Source: CAD feature listing. Evaluate the final solid. Frame: model axes, mm. A direction names the side the tool comes from. Coordinates: 2 decimals unless noted, no trailing zeros. Order: outer loops, then holes, each group sorted by start corner. A loop starts at its lowest first (then second) coordinate and runs counter-clockwise, first axis right, second up. Notation, with made-up numbers: (-10.75, -9) -> (28.25, -9) arc R20 cw to (28.25, 18) -> close; hole circle Ø10 at (-31.5, -36.5). An arc over 180 degrees is marked (long way). Put each result on its own line as item: value.
from build123d import *

# Parameters (mm, degrees)
BOSS_EXTRUDE1_DEPTH = 100
SKETCH2_R           = 10
CUT_EXTRUDE1_DEPTH  = 500
CUT_EXTRUDE2_DEPTH  = 500


with BuildPart() as part:
    # Sketch1 → Boss-Extrude1 (new body)
    with BuildSketch(Plane.XY):
        Polygon((0, 0), (100, 0), (100, -15), (-15, -15), (-15, 95), (100, 95), (100, 80), (0, 80), align=None)
    extrude(amount=BOSS_EXTRUDE1_DEPTH)

    # Sketch2 → Cut-Extrude1 (cut)
    with BuildSketch(Plane(origin=(0, 95, 0), x_dir=(1, 0, 0), z_dir=(0, 1, 0))):
        with Locations(Location((20, -25, 0), (0, 0, 270))):
            Circle(SKETCH2_R)
        with Locations(Location((70, -25, 0), (0, 0, 270))):
            Circle(SKETCH2_R)
        with Locations(Location((20, -75, 0), (0, 0, 270))):
            Circle(SKETCH2_R)
        with Locations(Location((70, -75, 0), (0, 0, 270))):
            Circle(SKETCH2_R)
    extrude(amount=-CUT_EXTRUDE1_DEPTH, mode=Mode.SUBTRACT)

    # Sketch3 → Cut-Extrude2 (cut)
    with BuildSketch(Plane(origin=(0, 0, 0), x_dir=(0, 0, -1), z_dir=(1, 0, 0))):
        with BuildLine():
            Line((-63.733404472, 53.788355895), (-44.717667379, 69.375025643))
            ThreePointArc((-44.717667379, 69.375025643), (-33.359667898, 68.249458127), (-34.485235414, 56.891458646))
            Line((-34.485235414, 56.891458646), (-53.500972507, 41.304788898))
            ThreePointArc((-53.500972507, 41.304788898), (-64.858971988, 42.430356414), (-63.733404472, 53.788355895))
        make_face()
        with BuildLine():
            Line((-51.188949328, 29.512455593), (-29.848080815, 53.133200052))
            ThreePointArc((-29.848080815, 53.133200052), (-17.387846498, 53.765023215), (-16.756023336, 41.304788898))
            Line((-16.756023336, 41.304788898), (-38.096891848, 17.684044439))
            ThreePointArc((-38.096891848, 17.684044439), (-50.557126165, 17.052221277), (-51.188949328, 29.512455593))
        make_face()
    extrude(amount=-CUT_EXTRUDE2_DEPTH, mode=Mode.SUBTRACT)


solid = part.part
1. Cut plane B-B on z = 75. Output: boundary loops of the cut face in (x, y), plus the area to 3 significant figures.
Numbers:
outline: (-15, -15) -> (10, -15) -> (10, 0) -> (0, 0) -> (0, 80) -> (10, 80) -> (10, 95) -> (-15, 95) -> close; (30, -15) -> (60, -15) -> (60, 0) -> (30, 0) -> close; (30, 80) -> (60, 80) -> (60, 95) -> (30, 95) -> close; (80, -15) -> (100, -15) -> (100, 0) -> (80, 0) -> close; (80, 80) -> (100, 80) -> (100, 95) -> (80, 95) -> close
area: 3,450 mm2
2. Set-up query: faces 1 (the cylindrical face through (23, 87.6, 34.54)), 2 (the flat face through (-7.395, 49.207, 43.86)), 3 (the flat face through (0, 41, 49)). Return all of +Z, -Z, +X, -X, +Y, -Y with unobstructed straight access to the full face (end or side cutting, diameter ignored); none if empty.
Numbers:
face 1: +Y, -Y
face 2: +X, -X
face 3: +Z, -Z, +X
3. Ray query, line 1 along X through (y, z) = (-12, 75); line 2 along Y through (x, z) = (51, 92); line 3 along X through (y, z) = (79, 23). Return the intervals inside material, ascending.
Numbers:
line 1: x = -15 to 10, 30 to 60, 80 to 100
line 2: y = -15 to 0, 80 to 95
line 3: x = -15 to 0
4. First-contact query: pin 1 (23 mm diameter, centred on x = 70, z = 25, fed in from +Y). Flat tip, straight axial feed; report the tip coordinate or a pass-through.
Numbers:
pin 1: stops at y = 95
5. Cut plane C-C on y = 49.5. Output: boundary loops of the cut face in (x, z).
Numbers:
outline: (-15, 0) -> (0, 0) -> (0, 14.78) -> (-15, 14.78) -> close; (-15, 33.13) -> (0, 33.13) -> (0, 43.5) -> (-15, 43.5) -> close; (-15, 66.45) -> (0, 66.45) -> (0, 100) -> (-15, 100) -> close
6. Cut plane A-A on x = 47.5. Output: boundary loops of the cut face in (y, z).
Numbers:
outline: (-15, 0) -> (0, 0) -> (0, 100) -> (-15, 100) -> close; (80, 0) -> (95, 0) -> (95, 100) -> (80, 100) -> close
7. Cut plane D-D on x = 13.5. Output: boundary loops of the cut face in (y, z), plus the area to 3 significant figures.
Numbers:
outline: (-15, 0) -> (0, 0) -> (0, 17.4) -> (-15, 17.4) -> close; (-15, 32.6) -> (0, 32.6) -> (0, 67.4) -> (-15, 67.4) -> close; (-15, 82.6) -> (0, 82.6) -> (0, 100) -> (-15, 100) -> close; (80, 0) -> (95, 0) -> (95, 17.4) -> (80, 17.4) -> close; (80, 32.6) -> (95, 32.6) -> (95, 67.4) -> (80, 67.4) -> close; (80, 82.6) -> (95, 82.6) -> (95, 100) -> (80, 100) -> close
area: 2,090 mm2
8. Pull-direction query (Y, two-part tool) for faces 4 (the flat face through (-7.395, 29.66, 27.277)), 5 (the flat face through (42, 95, 49)), 6 (the flat face through (-4, 36, 0)); classes: pulls with the +Y half, pulls with the -Y half, needs draft (parallel to the pull), parting line crosses it, or undercut.
Numbers:
face 4: undercut
face 5: pulls with the +Y half
face 6: needs draft
